Part print with two shaded views. Sizes in mm from the minimum x, y, z corner. Give positions to 0.01 mm unless a question says otherwise; leave off trailing zeros. Write each loop counter-clockwise with the first axis right and the second up, starting at its lowest first coordinate (ties: lowest second). Pieces come first, ordered by that corner, then holes. Notation, with made-up numbers: (16, -7) -> (57, -7) arc R8 cw to (57, 4) -> close; hole circle Ø2 at (40.25, -25). An arc over 180 degrees is marked (long way). Use one line per item in the form item = value. Start each with the question number.
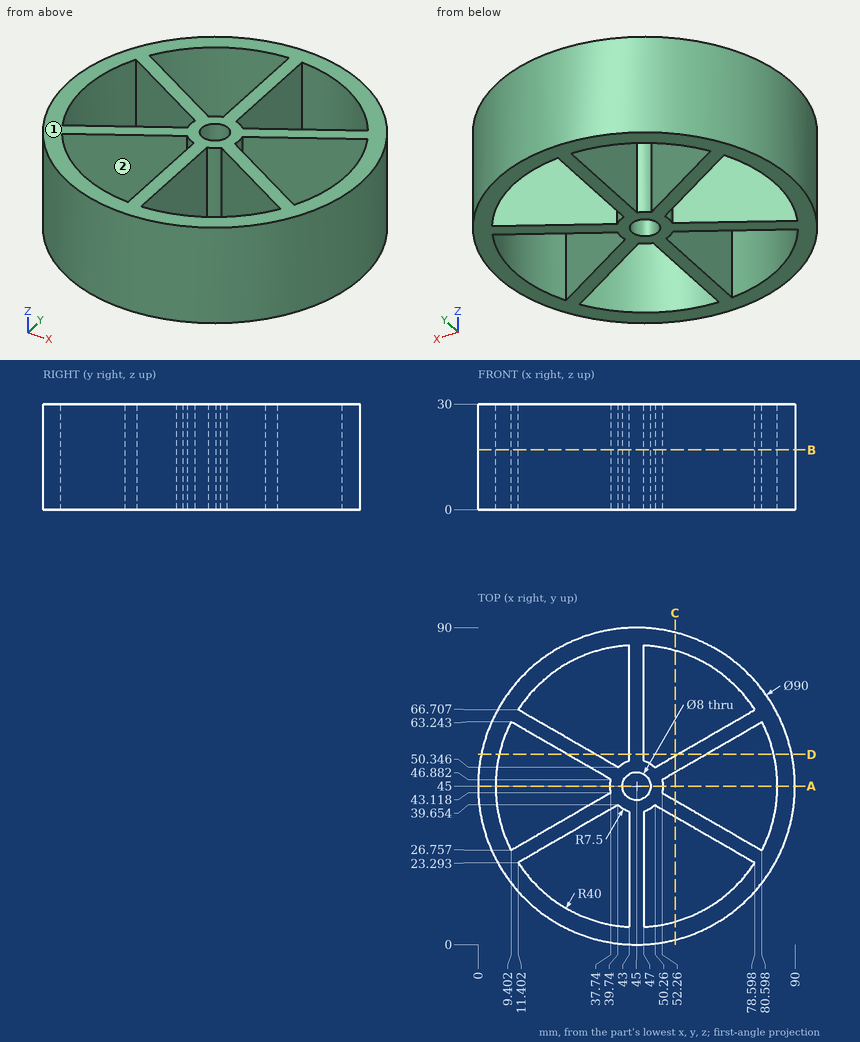
1) Two-plate mould, pull along Y, no slides. Class the marked faces 1 and 2: released by +Y, released by -Y, zero draft, split by the parting line, or undercut.
2) Cut at D-D (y = 54). Give the cut face in (x, z), and give its area (3 significant figures).
3) Cut at A-A (y = 45). Give the cut face in (x, z).
4) Cut at C-C (x = 56). Give the cut face in (y, z) (1 decimal).
5) Cut at B-B (z = 17). Give the cut face in (x, y), and give its area (3 significant figures).
6) Pin check, flat tips, straight feed: pin 1 (5 mm diameter, centred on y = 38.5, z = 22.5, fed in from +X); pin 2 (4 mm diameter, centred on y = 74, z = 9, fed in from +X); pin 3 (15 mm diameter, centred on y = 22, z = 18.5, fed in from -X). Stop position of each tip, or through.
7) Wall check: line 1 along Y through (x, z) = (71.5, 15); line 2 along Y through (x, z) = (45, 9.5); line 3 along Y through (x, z) = (73.5, 10.5) (1 decimal). Give the ranges that are in metal, low to high. Write a range as from..to.
Final values:
q1.face_1 = zero draft
q1.face_2 = undercut
q2.outline = (0.91, 0) -> (6.03, 0) -> (6.03, 30) -> (0.91, 30) -> close; (25.41, 0) -> (33.41, 0) -> (33.41, 30) -> (25.41, 30) -> close; (43, 0) -> (47, 0) -> (47, 30) -> (43, 30) -> close; (56.59, 0) -> (64.59, 0) -> (64.59, 30) -> (56.59, 30) -> close; (83.97, 0) -> (89.09, 0) -> (89.09, 30) -> (83.97, 30) -> close
q2.area = 907 mm^2
q3.outline = (0, 0) -> (5, 0) -> (5, 30) -> (0, 30) -> close; (37.5, 0) -> (41, 0) -> (41, 30) -> (37.5, 30) -> close; (49, 0) -> (52.5, 0) -> (52.5, 30) -> (49, 30) -> close; (85, 0) -> (90, 0) -> (90, 30) -> (85, 30) -> close
q4.outline = (1.4, 0) -> (6.5, 0) -> (6.5, 30) -> (1.4, 30) -> close; (36.3, 0) -> (41, 0) -> (41, 30) -> (36.3, 30) -> close; (49, 0) -> (53.7, 0) -> (53.7, 30) -> (49, 30) -> close; (83.5, 0) -> (88.6, 0) -> (88.6, 30) -> (83.5, 30) -> close
q5.outline = circle Ø90 at (45, 45); hole (9.4, 26.76) -> (37.74, 43.12) arc R7.5 cw to (37.74, 46.88) -> (9.4, 63.24) arc R40 ccw to start; hole (11.4, 23.29) arc R40 ccw to (43, 5.05) -> (43, 37.77) arc R7.5 cw to (39.74, 39.65) -> close; hole (11.4, 66.71) -> (39.74, 50.35) arc R7.5 cw to (43, 52.23) -> (43, 84.95) arc R40 ccw to start; hole circle Ø8 at (45, 45); hole (47, 5.05) arc R40 ccw to (78.6, 23.29) -> (50.26, 39.65) arc R7.5 cw to (47, 37.77) -> close; hole (47, 52.23) arc R7.5 cw to (50.26, 50.35) -> (78.6, 66.71) arc R40 ccw to (47, 84.95) -> close; hole (52.26, 43.12) -> (80.6, 26.76) arc R40 ccw to (80.6, 63.24) -> (52.26, 46.88) arc R7.5 cw to start
q5.area = 2,240 mm^2
q6.pin_1 = 89.82
q6.pin_2 = 81
q6.pin_3 = 2.75
q7.line_1 = 8.63..15.04, 27.39..32.01, 57.99..62.61, 74.96..81.37
q7.line_2 = 0..41, 49..90
q7.line_3 = 10.2..16.9, 26.2..30.9, 59.1..63.8, 73.1..79.8
